Geometry: final body of the model. Coordinates: model frame, mm. Face numbers are marked on the shaded views. A direction names the side the tool comes from. Round coordinates to 2 decimals unless told otherwise and drop trailing zeros. Loops run counter-clockwise (first coordinate to the right, second up) from the corner with the lowest first, then second, coordinate; pieces in that order, holes last. Notation, with made-up numbers: M 80,45 L 131,45 A18 ccw 131,62 Z; hole C 54.5,3 d1. An arc over 180 degrees is marked long. Answer as a JSON object with one key per item and string values.
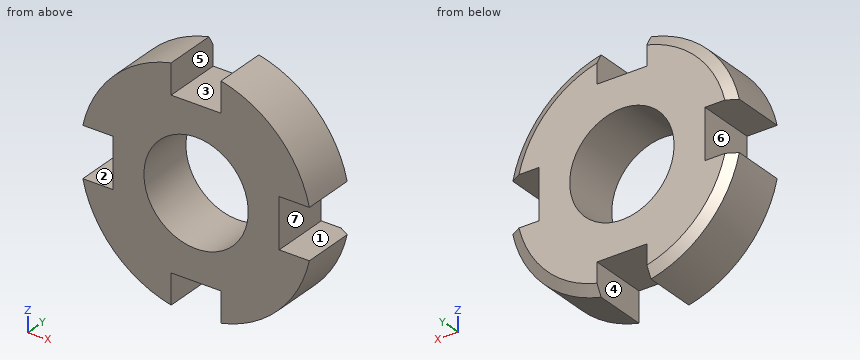
```python
from build123d import *
from OCP.BRepFilletAPI import BRepFilletAPI_MakeChamfer

# Parameters (mm, degrees)
EXTRUDE_1_DEPTH = 5
M10X1_0_1_D     = 9
CHAMFER_1_SIZE  = 0.5
CHAMFER_1_SIZE2 = 0.866025404


with BuildPart() as part:
    # 草图1 → 凸台-拉伸1 (new body)
    with BuildSketch(Plane(origin=(0, 0, 0), x_dir=(1, 0, 0), z_dir=(0, 1, 0))):
        with BuildLine():
            Line((-2.15, 9.766140486), (-2.15, 7.166140486))
            Line((-2.15, 7.166140486), (2.15, 7.166140486))
            Line((2.15, 7.166140486), (2.15, 9.766140486))
            ThreePointArc((2.15, 9.766140486), (7.071067812, 7.071067812), (9.766140486, 2.15))
            Line((9.766140486, 2.15), (7.166140486, 2.15))
            Line((7.166140486, 2.15), (7.166140486, -2.15))
            Line((7.166140486, -2.15), (9.766140486, -2.15))
            ThreePointArc((9.766140486, -2.15), (7.071067812, -7.071067812), (2.15, -9.766140486))
            Line((2.15, -9.766140486), (2.15, -7.166140486))
            Line((2.15, -7.166140486), (-2.15, -7.166140486))
            Line((-2.15, -7.166140486), (-2.15, -9.766140486))
            ThreePointArc((-2.15, -9.766140486), (-7.071067812, -7.071067812), (-9.766140486, -2.15))
            Line((-9.766140486, -2.15), (-7.166140486, -2.15))
            Line((-7.166140486, -2.15), (-7.166140486, 2.15))
            Line((-7.166140486, 2.15), (-9.766140486, 2.15))
            ThreePointArc((-9.766140486, 2.15), (-7.071067812, 7.071067812), (-2.15, 9.766140486))
        make_face()
    extrude(amount=EXTRUDE_1_DEPTH)

    # M10x1.0 螺纹孔1 (through all)
    with Locations(Plane(origin=(0, 5, 0), x_dir=(1, 0, 0), z_dir=(0, 1, 0))):
        with Locations((0, 0)):
            Hole(M10X1_0_1_D / 2)

    # 倒角1: one chamfer whose edges measure the first distance from different faces: ONE call of the kernel's chamfer builder (chamfer() names one face for all edges)
    chamfer_1_edges_1 = [part.edges().sort_by_distance(p)[0] for p in [
        (-7.071067812, 5, 7.071067812),
    ]]
    chamfer_1_side_1 = [part.faces().sort_by_distance(p)[0] for p in [
        (-7.071067812, 2.5, 7.071067812),
    ]]
    chamfer_1_edges_2 = [part.edges().sort_by_distance(p)[0] for p in [
        (7.071067812, 5, 7.071067812),
    ]]
    chamfer_1_side_2 = [part.faces().sort_by_distance(p)[0] for p in [
        (7.071067812, 2.5, 7.071067812),
    ]]
    chamfer_1_edges_3 = [part.edges().sort_by_distance(p)[0] for p in [
        (-7.071067812, 5, -7.071067812),
    ]]
    chamfer_1_side_3 = [part.faces().sort_by_distance(p)[0] for p in [
        (-7.071067812, 2.5, -7.071067812),
    ]]
    chamfer_1_edges_4 = [part.edges().sort_by_distance(p)[0] for p in [
        (7.071067812, 5, -7.071067812),
    ]]
    chamfer_1_side_4 = [part.faces().sort_by_distance(p)[0] for p in [
        (7.071067812, 2.5, -7.071067812),
    ]]
    chamfer_1 = BRepFilletAPI_MakeChamfer(part.part.solid().wrapped)
    for e in chamfer_1_edges_1:
        chamfer_1.Add(CHAMFER_1_SIZE, CHAMFER_1_SIZE2, e.wrapped, chamfer_1_side_1[0].wrapped)  # the first distance lies on this face
    for e in chamfer_1_edges_2:
        chamfer_1.Add(CHAMFER_1_SIZE, CHAMFER_1_SIZE2, e.wrapped, chamfer_1_side_2[0].wrapped)  # the first distance lies on this face
    for e in chamfer_1_edges_3:
        chamfer_1.Add(CHAMFER_1_SIZE, CHAMFER_1_SIZE2, e.wrapped, chamfer_1_side_3[0].wrapped)  # the first distance lies on this face
    for e in chamfer_1_edges_4:
        chamfer_1.Add(CHAMFER_1_SIZE, CHAMFER_1_SIZE2, e.wrapped, chamfer_1_side_4[0].wrapped)  # the first distance lies on this face
    add(Compound.cast(chamfer_1.Shape()), mode=Mode.REPLACE)


solid = part.part
```
1) Pull-direction query (Z, two-part tool) for the marked faces 1, 2, 3 and 4; classes: +Z half, -Z half, draft (parallel to the pull), parting line (faces both ways), or undercut.
Geometry results:
{"face 1": "undercut", "face 2": "undercut", "face 3": "+Z half", "face 4": "draft"}
2) Cut plane A-A on x = 0. Return the cut outline in (y, z), and give its area (3 significant figures).
Geometry results:
{"outline": "M 0,-7.17 L 5,-7.17 L 5,-4.5 L 0,-4.5 Z; M 0,4.5 L 5,4.5 L 5,7.17 L 0,7.17 Z", "area": "26.7 mm2"}
3) Line query: probe 1 along Z at (x, y) = (0, 2.45); probe 2 along Z at (x, y) = (-4, 4.1); probe 3 along X at (y, z) = (2.85, -2.5). Output: solid intervals per line, ascending.
Geometry results:
{"probe 1": "-7.17 to -4.5, 4.5 to 7.17", "probe 2": "-9.17 to -2.06, 2.06 to 9.17", "probe 3": "-9.68 to -3.74, 3.74 to 9.68"}
4) First-contact query: pin 1 (1.3 mm diameter, centred on x = 0.5, y = 1.5, fed in from +Z); pin 2 (1.3 mm diameter, centred on y = 3.5, z = 0, fed in from +X); pin 3 (5.5 mm diameter, centred on x = 0, z = 0, fed in from -Y); pin 4 (0.8 mm diameter, centred on y = 3.5, z = 8.5, fed in from +X). Flat tips, straight axial feed; report the tip coordinate or a pass-through.
Geometry results:
{"pin 1": "z = 7.17", "pin 2": "x = 7.17", "pin 3": "through", "pin 4": "x = 5.86"}
5) Cut plane C-C on y = 2.2. Return the cut outline in (x, z), and give its area (3 significant figures).
Geometry results:
{"outline": "M -9.77,-2.15 A10 ccw -2.15,-9.77 L -2.15,-7.17 L 2.15,-7.17 L 2.15,-9.77 A10 ccw 9.77,-2.15 L 7.17,-2.15 L 7.17,2.15 L 9.77,2.15 A10 ccw 2.15,9.77 L 2.15,7.17 L -2.15,7.17 L -2.15,9.77 A10 ccw -9.77,2.15 L -7.17,2.15 L -7.17,-2.15 Z; hole C 0,0 d9", "area": "203 mm2"}
6) Cut plane B-B on z = 0. Return the cut outline in (x, y), and give its area (3 significant figures).
Geometry results:
{"outline": "M -7.17,0 L -4.5,0 L -4.5,5 L -7.17,5 Z; M 4.5,0 L 7.17,0 L 7.17,5 L 4.5,5 Z", "area": "26.7 mm2"}
7) Set-up query: the marked faces 5, 6 and 7. Return all of +Z, -Z, +X, -X, +Y, -Y with unobstructed straight access to the full face (end or side cutting, diameter ignored); none if empty.
Geometry results:
{"face 5": "+Z, +Y, -Y", "face 6": "-X, +Y, -Y", "face 7": "+X, +Y, -Y"}
